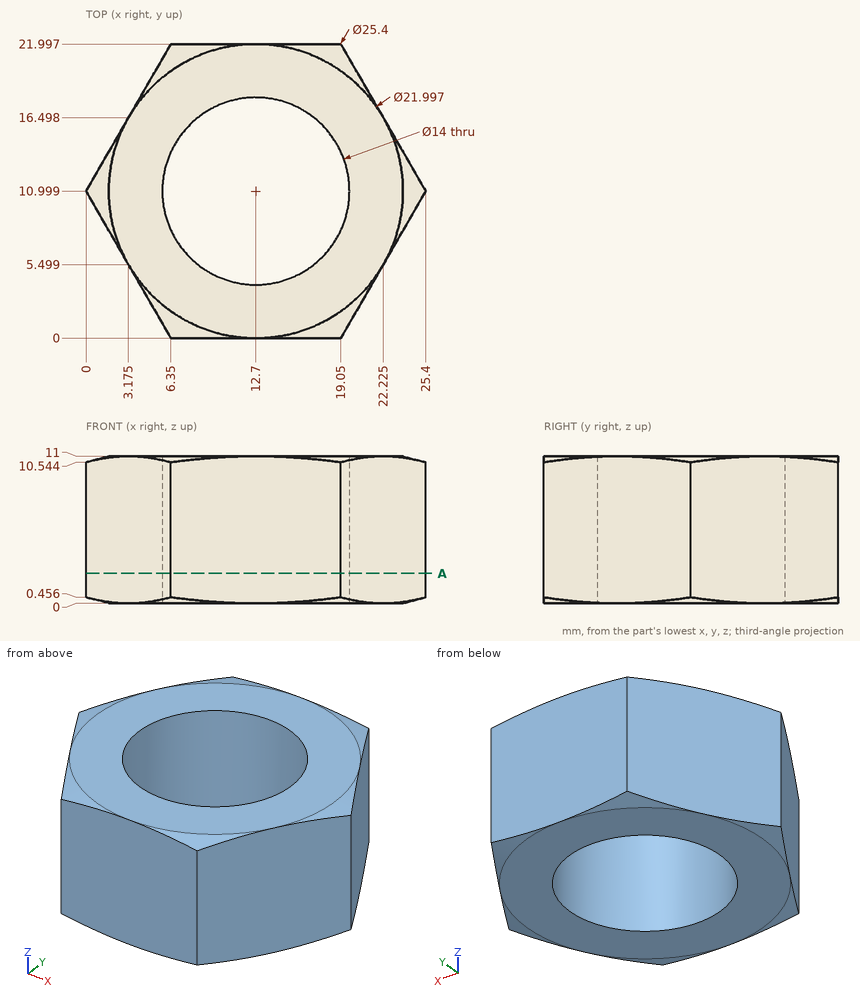
Print and shaded views of the part. All mm, measured from the part's lowest x, y and z. Round coordinates to 2 decimals unless told otherwise and drop trailing zeros. Write each loop counter-clockwise with the first axis right and the second up, starting at its lowest first coordinate (ties: lowest second). Pieces come first, ordered by that corner, then holes. Notation, with made-up numbers: (48.5, 53.5) - (99.5, 53.5) arc R38 cw to (99.5, 91.5) - close; hole circle Ø11 at (43.25, 76.25). An arc over 180 degrees is marked (long way). Write each question's results on one line, items separated by ' | '. Start each with the question number.
Item 1: Wall check: L1, parallel to Y at x = 12.25, z = 7 (1 decimal); L2, parallel to Y at x = 11.5, z = 3 (1 decimal); L3, parallel to X at y = 14, z = 8 (1 decimal). Give the ranges that are in metal, low to high. Write a range as [from, to].
Item 2: Saw through at A-A (z = 2.25). Write the cut outline in (x, y).
Item 3: Drop flat-ended pins along their axis: P1, Ø4, axis at y = 8.5, z = 6.5, coming from the +X side; P2, Ø1, axis at x = 22, z = 5.5, coming from the -Y side (1 decimal). Give the stop position or say it passes through.
Results are:
1) L1: y = [0, 4], [18, 22] | L2: y = [0, 4.1], [17.9, 22] | L3: x = [1.7, 6.4], [19, 23.7]
2) outline: (0, 11) - (6.35, 0) - (19.05, 0) - (25.4, 11) - (19.05, 22) - (6.35, 22) - close; hole circle Ø14 at (12.7, 11)
3) P1: stops at x = 25.11 | P2: stops at y = 4.2
